Can you work these out from the model? Positions are in its coordinate system, mm. A direction names the side the tool comes from. Coordinates: 2 decimals unless noted, no trailing zeros. Order: outer loops, then holes, each group sorted by start corner. A loop starts at its lowest first (then second) coordinate and runs counter-clockwise, first axis right, second up. Notation, with made-up numbers: (11.25, -21.5) -> (64.25, -21.5) arc R19 ccw to (64.25, 11.5) -> close; hole circle Ø2 at (-2, -33.5). An arc over 180 degrees is marked (long way). Return JSON: item names as keys, results as strings. Group by question number.
1) If we section it at C-C, the plane z = 72.5: Please give me the cut outline in (x, y).
2) If I drill on probe 1 along Z at (x, y) = (-2.25, -36.5); probe 2 along X at (y, z) = (-36, -13); probe 3 along Y at (x, z) = (-7, 60), over which ranges is the centre line in solid material (lowest first)? Write a range as from..to.
3) Thinking about a two-plate mould opening in Z: for faces 1 (the flat face through (7, -23, -5)), 2 (the flat face through (0, -19, 95)), 3 (the cylindrical face through (0.14, -49.97, 1.5)), 4 (the flat face through (0, -51.399, 35)), which applies, +Z half, -Z half, draft (parallel to the pull), parting line (faces both ways), or undercut?
4) For faces 5 (the flat face through (-7, -23, 86)), 6 (the cylindrical face through (0.14, -49.9, 68.57)), 7 (the flat face through (7, -36, 75)), which set-ups out of +Z, -Z, +X, -X, +Y, -Y let a thin tool reach every point of the face, with its end or its side?
5) If we section it at B-B, the plane y = -36.5: Please give me the cut outline in (x, z), then the cut area to 3 significant figures.
6) If we section it at A-A, the plane y = -21.5: Please give me the cut outline in (x, z).
7) For pin 1 (6.5 mm diameter, centred on x = 5.5, z = 83, fed in from -Y); pin 2 (5 mm diameter, centred on x = 0, y = -71.5, fed in from -Z); pin 3 (1.5 mm diameter, centred on x = 7.5, z = 76.5, fed in from +Y), each with a flat end and sliding along its axis, tell me the tip position at first contact or that it passes through.
8) If we section it at D-D, the plane z = 59.5: Please give me the cut outline in (x, y), then the cut area to 3 significant figures.
from build123d import *

# Parameters (mm, degrees)
FRAME_PLATE_8MM_DEPTH      = 4
FRAME_RIM_8MM_DEPTH        = 4
FRAME_FLANGE_20MM_DEPTH    = 10
SCREW_BOSS_DEPTH           = 25
RELIEF_CHANNEL_CUT_DEPTH   = 25
M12X1_5_TAPPED_HOLE1_D     = 12
M12X1_5_TAPPED_HOLE1_DEPTH = 25
EDGE_FILLET_R2_R           = 2


with BuildPart() as part:
    # Frame Profile Sketch → Frame Plate 8mm (new, symmetric)
    with BuildSketch(Plane(origin=(0, 0, 0), x_dir=(0, 0, -1), z_dir=(1, 0, 0))):
        with BuildLine():
            ThreePointArc((-65, -81), (-86.213203436, -72.213203436), (-95, -51))
            Line((-95, -51), (-95, 0))
            Line((-95, 0), (-75, 0))
            Line((-75, 0), (-75, -46.399278983))
            ThreePointArc((-75, -46.399278983), (-72.071067812, -53.470346795), (-65, -56.399278983))
            Line((-65, -56.399278983), (-5, -56.399278983))
            ThreePointArc((-5, -56.399278983), (2.071067812, -53.470346795), (5, -46.399278983))
            Line((5, -46.399278983), (5, 0))
            Line((5, 0), (25, -13))
            Line((25, -13), (25, -51))
            ThreePointArc((25, -51), (16.213203436, -72.213203436), (-5, -81))
            Line((-5, -81), (-65, -81))
        make_face()
    extrude(amount=FRAME_PLATE_8MM_DEPTH, both=True)

    # Sketch1_3 → Frame Rim 8mm (add, symmetric)
    with BuildSketch(Plane(origin=(0, 0, 0), x_dir=(0, 0, -1), z_dir=(1, 0, 0))):
        with BuildLine():
            ThreePointArc((-65, -56.399278983), (-72.071067812, -53.470346795), (-75, -46.399278983))
            Line((-75, -46.399278983), (-75, 0))
            Line((-75, 0), (-70, 0))
            Line((-70, 0), (-70, -46.399278983))
            ThreePointArc((-70, -46.399278983), (-68.535533906, -49.934812889), (-65, -51.399278983))
            Line((-65, -51.399278983), (-5, -51.399278983))
            ThreePointArc((-5, -51.399278983), (-1.464466094, -49.934812889), (0, -46.399278983))
            Line((0, -46.399278983), (0, 0))
            Line((0, 0), (5, 0))
            Line((5, 0), (5, -46.399278983))
            ThreePointArc((5, -46.399278983), (2.071067812, -53.470346795), (-5, -56.399278983))
            Line((-5, -56.399278983), (-65, -56.399278983))
        make_face()
    extrude(amount=FRAME_RIM_8MM_DEPTH, both=True)

    # Sketch1_4 → Frame Flange 20mm (add, symmetric)
    with BuildSketch(Plane(origin=(0, 0, 0), x_dir=(0, 0, -1), z_dir=(1, 0, 0))):
        with BuildLine():
            ThreePointArc((-65, -56.399278983), (-72.071067812, -53.470346795), (-75, -46.399278983))
            Line((-75, -46.399278983), (-75, 0))
            Line((-75, 0), (-70, 0))
            Line((-70, 0), (-70, -46.399278983))
            ThreePointArc((-70, -46.399278983), (-68.535533906, -49.934812889), (-65, -51.399278983))
            Line((-65, -51.399278983), (-5, -51.399278983))
            ThreePointArc((-5, -51.399278983), (-1.464466094, -49.934812889), (0, -46.399278983))
            Line((0, -46.399278983), (0, 0))
            Line((0, 0), (5, 0))
            Line((5, 0), (5, -46.399278983))
            ThreePointArc((5, -46.399278983), (2.071067812, -53.470346795), (-5, -56.399278983))
            Line((-5, -56.399278983), (-65, -56.399278983))
        make_face()
    extrude(amount=FRAME_FLANGE_20MM_DEPTH, both=True)

    # Screw Boss Sketch → Screw Boss (add)
    with BuildSketch(Plane.XY.offset(95)):
        with BuildLine():
            Line((-10, -10), (-10, -23))
            Line((-10, -23), (10, -23))
            Line((10, -23), (10, -10))
            ThreePointArc((10, -10), (0, 0), (-10, -10))
        make_face()
    extrude(amount=-SCREW_BOSS_DEPTH)

    # Relief Channel Sketch → Relief Channel Cut (cut)
    with BuildSketch(Plane.XY.offset(95)):
        with BuildLine():
            Line((-10, 0), (-4, 0))
            Line((-4, 0), (-4, -0.83484861))
            ThreePointArc((-4, -0.83484861), (-8.366600265, -4.522774425), (-10, -10))
            Line((-10, -10), (-10, 0))
        make_face()
        with BuildLine():
            Line((-4, 0), (-4, -0.83484861))
            ThreePointArc((-4, -0.83484861), (-2.043096424, -0.210936868), (2.7e-08, 0))
            Line((2.7e-08, 0), (-4, 0))
        make_face()
        with BuildLine():
            Line((4, 0), (2.7e-08, 0))
            ThreePointArc((2.7e-08, 0), (2.04309645, -0.210936873), (4, -0.83484861))
            Line((4, -0.83484861), (4, 0))
        make_face()
        with BuildLine():
            Line((10, -10), (10, 0))
            Line((10, 0), (4, 0))
            Line((4, 0), (4, -0.83484861))
            ThreePointArc((4, -0.83484861), (8.366600265, -4.522774425), (10, -10))
        make_face()
    extrude(amount=-RELIEF_CHANNEL_CUT_DEPTH, mode=Mode.SUBTRACT)

    # M12x1.5 Tapped Hole1
    with Locations(Plane.XY.offset(95)):
        with Locations((0, -10)):
            Hole(M12X1_5_TAPPED_HOLE1_D / 2, depth=M12X1_5_TAPPED_HOLE1_DEPTH)

    # Edge Fillet R2
    edge_fillet_r2_edges = [part.edges().sort_by_distance(p)[0] for p in [
        (-7, -23, 75),
        (7, -23, 75),
    ]]
    fillet(edge_fillet_r2_edges, radius=EDGE_FILLET_R2_R)


solid = part.part
Result sheet:
{
 "1": {"outline": "(-10, -53.01) -> (-4, -53.01) -> (-4, -80.05) -> (4, -80.05) -> (4, -53.01) -> (10, -53.01) -> (10, -10) arc R10 ccw to (-10, -10) -> close; hole circle Ø12 at (0, -10)"},
 "2": {"probe 1": "z = -25..0, 70..95", "probe 2": "x = -4..4", "probe 3": "y = -56.4..-51.4"},
 "3": {"face 1": "-Z half", "face 2": "+Z half", "face 3": "undercut", "face 4": "undercut"},
 "4": {"face 5": "+Z, -X, -Y", "face 6": "+X, -X, +Y", "face 7": "+Z, +X, -Y"},
 "5": {"outline": "(-10, -5) -> (-4, -5) -> (-4, -25) -> (4, -25) -> (4, -5) -> (10, -5) -> (10, 0) -> (-10, 0) -> close; (-10, 70) -> (10, 70) -> (10, 75) -> (4, 75) -> (4, 95) -> (-4, 95) -> (-4, 75) -> (-10, 75) -> close", "area": "520 mm2"},
 "6": {"outline": "(-10, -5) -> (-4, -5) -> (-4, -25) -> (4, -25) -> (4, -5) -> (10, -5) -> (10, 0) -> (-10, 0) -> close; (-10, 70) -> (10, 70) -> (10, 95) -> (-10, 95) -> close"},
 "7": {"pin 1": "stops at y = -76.91", "pin 2": "stops at z = -19", "pin 3": "stops at y = -2.62"},
 "8": {"outline": "(-10, -56.4) -> (-4, -56.4) -> (-4, -81) -> (4, -81) -> (4, -56.4) -> (10, -56.4) -> (10, -51.4) -> (-10, -51.4) -> close", "area": "297 mm2"}
}
